Source: CAD feature listing. Evaluate the final solid. Frame: model axes, mm. A direction names the side the tool comes from. Round coordinates to 2 decimals unless told otherwise and drop trailing zeros. Order: outer loops, then holes, each group sorted by start corner. A loop starts at its lowest first (then second) coordinate and runs counter-clockwise, first axis right, second up. Notation, with made-up numbers: M -29.75,66 L 18.25,66 A9 cw 18.25,78 Z; hole C 42,59 d11. An arc over 180 degrees is marked long. Answer in a Markdown table with one row per item. Add a question column.
```python
from build123d import *

# Parameters (mm, degrees)
SKETCH_1_R          = 10
EXTRUDE_1_DEPTH     = 200
SKETCH_2_OUTSIDE_W  = 62.398
SKETCH_2_OUTSIDE_H  = 62.398
SKETCH_2_OUTSIDE_R  = 4
CUT_EXTRUDE_1_DEPTH = 20
CHAMFER_1_SIZE      = 0.5


with BuildPart() as part:
    # 草图1 → 凸台-拉伸1 (new body)
    with BuildSketch(Plane.XY):
        Circle(SKETCH_1_R)
    extrude(amount=EXTRUDE_1_DEPTH)

    # 草图2 outside → 切除-拉伸1 (cut)
    with BuildSketch(Plane(origin=(0, 0, 0), x_dir=(-1, 0, 0), z_dir=(0, 0, -1))):
        Rectangle(SKETCH_2_OUTSIDE_W, SKETCH_2_OUTSIDE_H)
        Circle(SKETCH_2_OUTSIDE_R, mode=Mode.SUBTRACT)
    extrude(amount=-CUT_EXTRUDE_1_DEPTH, mode=Mode.SUBTRACT)

    # 倒角1
    chamfer_1_edges = [part.edges().sort_by_distance(p)[0] for p in [
        (4, 0, 0),
        (-10, 0, 200),
        (-10, 0, 20),
    ]]
    chamfer(chamfer_1_edges, length=CHAMFER_1_SIZE)


solid = part.part
```
(1) Access query for faces 1 (the face through (-2, -4, 20)), 2 (the face through (-2.17, -9.76, 108.75)). Directions: +Z, -Z, +X, -X, +Y, -Y. A direction counts if a zero-diameter tool reaches every point of the face in a straight line with its end or side. Return the directions, or none.
(2) Line query: line 1 (Y direction, x = 0.25, z = 103.5); line 2 (Z direction, x = -3.5, y = 3); line 3 (X direction, y = 0.5, z = 18). Output: solid intervals per line, ascending. Write a range as from..to.
(3) Cut plane D-D (z = 14.5). Return loops of the section in (x, y).
(4) Cut plane A-A (y = 0). Return loops of the section in (x, z).
(5) Pin query (flat end, axial travel): pin 1 (1 mm diameter, centred on x = 8, z = 53, fed in from -Y); pin 2 (3 mm diameter, centred on x = -3, y = 5, fed in from -Z); pin 3 (4 mm diameter, centred on x = 4, z = 92, fed in from +Y). Return the tip coordinate at first contact, or that it passes through.
(6) Cut plane C-C (z = 173). Return loops of the section in (x, y).
Answer list:
| question | item | result |
|---|---|---|
| 1 | face 1 | -Z |
| 1 | face 2 | +Z, -Z |
| 2 | line 1 | -10..10 |
| 2 | line 2 | 20..200 |
| 2 | line 3 | -3.97..3.97 |
| 3 | outline | C 0,0 d8 |
| 4 | outline | M -10,20.5 L -9.5,20 L -4,20 L -4,0.5 L -3.5,0 L 3.5,0 L 4,0.5 L 4,20 L 9.5,20 L 10,20.5 L 10,199.5 L 9.5,200 L -9.5,200 L -10,199.5 Z |
| 5 | pin 1 | y = -6.61 |
| 5 | pin 2 | z = 20 |
| 5 | pin 3 | y = 9.8 |
| 6 | outline | C 0,0 d20 |
